Can you work these out from the drawing? Everything is in mm from the part's minimum corner. A direction names the side the tool comes from. Give positions to 0.01 mm unless a question says otherwise; leave off trailing zeros. Loops run counter-clockwise (first coordinate to the right, second up) from the corner with the lowest first, then second, coordinate; pieces in that order, holes last. Notation, with made-up numbers: (63, -18) -> (90, -18) arc R18 ccw to (90, -1) -> close; hole circle Ø8 at (52, 16.25). An arc over 180 degrees is marked (long way). Return JSON: item names as keys, results as strings. Group by question number.
Q1. Suppose I cut it at D-D, the plane z = 45. Please give me the cut outline in (x, y).
Q2. Will these pins go through, and if not, where does the flat tip stop? pin 1 (3 mm diameter, centred on x = 58, z = 33, fed in from +Y); pin 2 (2 mm diameter, centred on x = 18, z = 26, fed in from -Y); pin 3 (10 mm diameter, centred on y = 45.5, z = 19.5, fed in from -X); pin 4 (12 mm diameter, centred on x = 19, z = 59, fed in from -Y).
Q3. Suppose I cut it at C-C, the plane x = 43. Please give me the cut outline in (y, z).
Q4. Thinking about a two-plate mould opening in Z: for the marked faces 1, 2 and 3, which applies, pulls with the +Z half, pulls with the -Z half, needs draft (parallel to the pull), parting line crosses it, or undercut?
Q5. Which directions (+Z, -Z, +X, -X, +Y, -Y) give clear straight access to the entire face, cutting with the end or side of a thin tool? Please do the marked faces 4, 5, 6, 7 and 8.
Q6. Suppose I cut it at B-B, the plane z = 62. Please give me the cut outline in (x, y) (1 decimal).
Q7. Suppose I cut it at A-A, the plane y = 19. Please give me the cut outline in (x, z), and give its area (3 significant figures).
Q8. I need wall thicknesses on line 1 along X through (y, z) = (38, 69.5); line 2 along Z through (x, y) = (51.5, 61.5); line 3 along Z through (x, y) = (59, 67). Which ranges of each line are inside material? Lowest first, please. Write a range as [from, to].
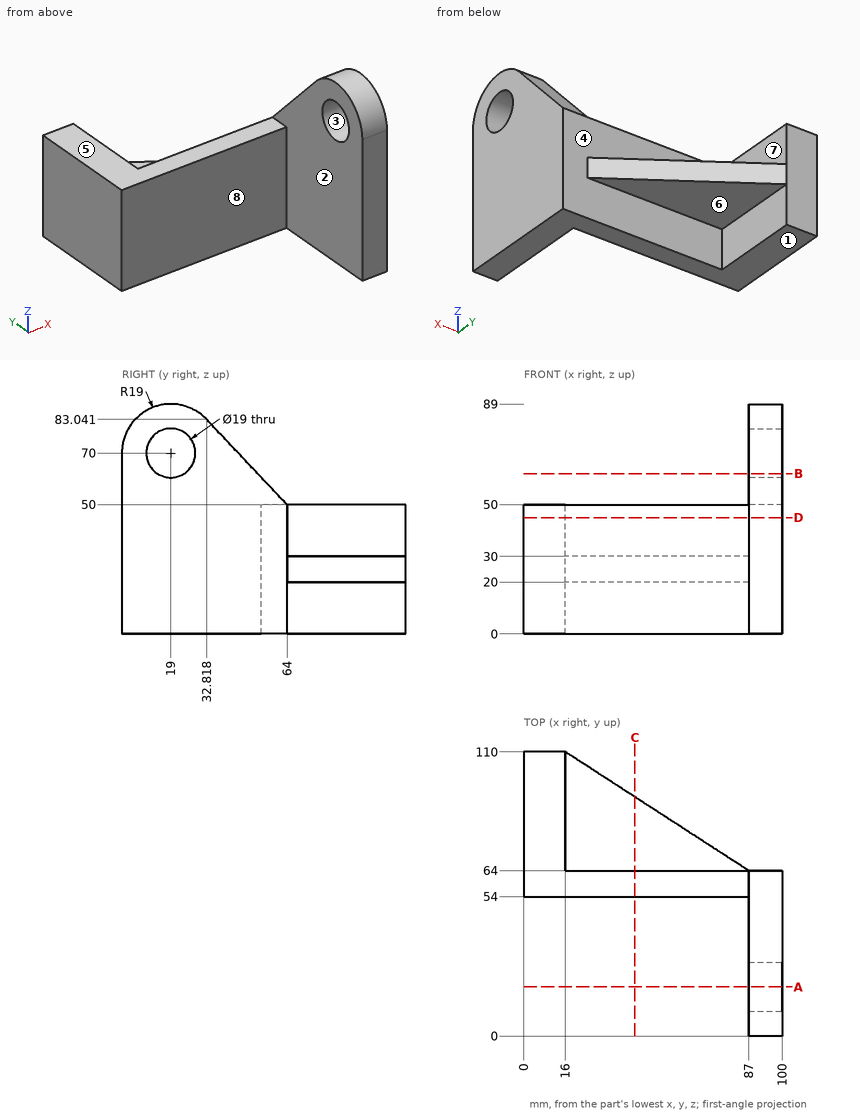
Ans:
{
 "1": {"outline": "(0, 54) -> (87, 54) -> (87, 0) -> (100, 0) -> (100, 64) -> (16, 64) -> (16, 110) -> (0, 110) -> close"},
 "2": {"pin 1": "stops at y = 64", "pin 2": "stops at y = 54", "pin 3": "stops at x = 87", "pin 4": "passes through"},
 "3": {"outline": "(54, 0) -> (64, 0) -> (64, 20) -> (92.51, 20) -> (92.51, 30) -> (64, 30) -> (64, 50) -> (54, 50) -> close"},
 "4": {"face 1": "pulls with the -Z half", "face 2": "needs draft", "face 3": "undercut"},
 "5": {"face 4": "+X, +Y", "face 5": "+Z, -X, +Y, -Y", "face 6": "-Z, +X, +Y", "face 7": "+Z, +X, +Y", "face 8": "+Z, -Z, -X, -Y"},
 "6": {"outline": "(87, 0) -> (100, 0) -> (100, 13.9) -> (87, 13.9) -> close; (87, 24.1) -> (100, 24.1) -> (100, 52.7) -> (87, 52.7) -> close"},
 "7": {"outline": "(87, 0) -> (100, 0) -> (100, 60.5) -> (87, 60.5) -> close; (87, 79.5) -> (100, 79.5) -> (100, 89) -> (87, 89) -> close", "area": "910 mm^2"},
 "8": {"line 1": "x = [87, 100]", "line 2": "z = [0, 50]", "line 3": "z = [20, 30]"}
}
